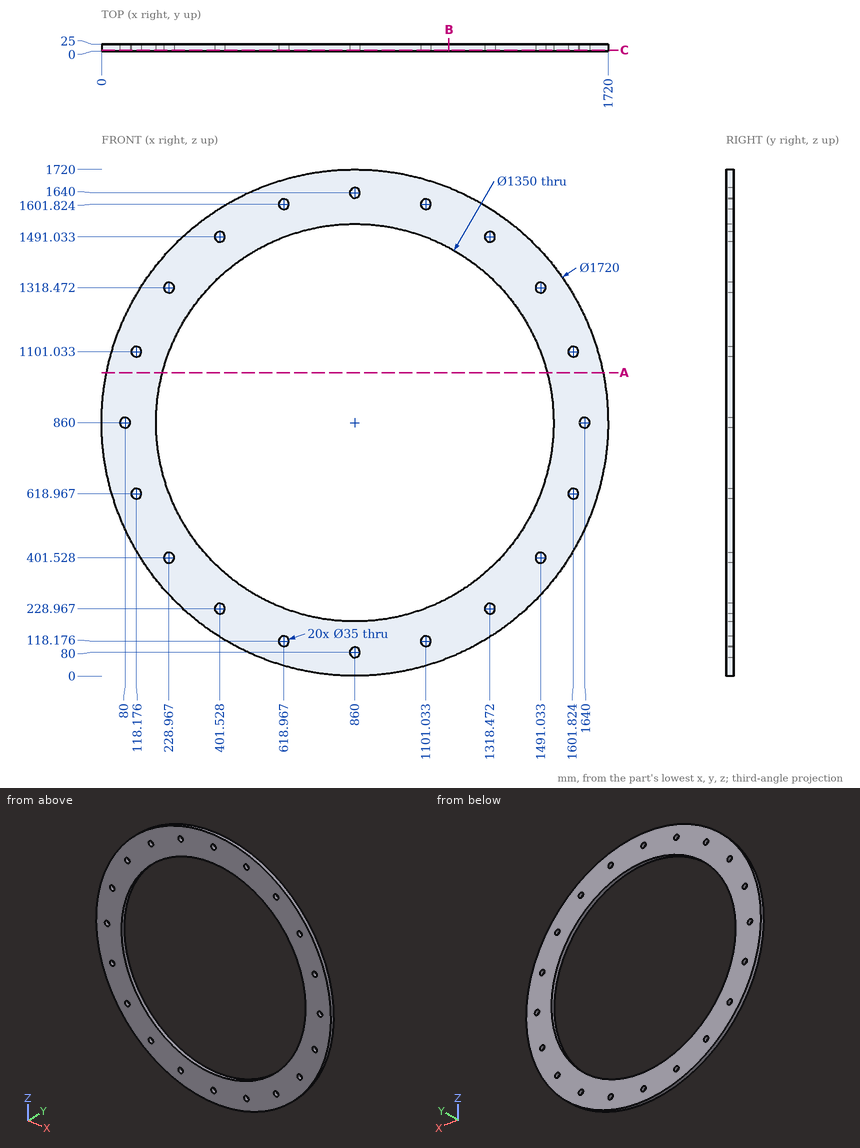
Geometry: see drawing. Coordinates: mm, zero at the bounding-box minimum. Coordinates: 2 decimals unless noted, no trailing zeros. Write each loop counter-clockwise with the first axis right and the second up, starting at its lowest first coordinate (ties: lowest second). Pieces come first, ordered by that corner, then holes. Notation, with made-up numbers: M 36.25,14.5 L 77.25,14.5 A25 ccw 77.25,26.5 Z; hole C 76,36.25 d3. An arc over 180 degrees is marked long. Answer as a JSON object with one key per item and string values.
1. Cut plane C-C on y = 4.25. State how many separate pieces and enclosed holes the cut face has, plus the area to 3 significant figures.
Evaluation:
{"separate pieces": "1", "enclosed holes": "21", "area": "873,000 mm^2"}
2. Ray query, L1, parallel to X at y = 15.25, z = 860; L2, parallel to Z at x = 878, y = 6.75; L3, parallel to Z at x = 1208, y = 9.75 (1 decimal). Return the intervals inside material, ascending.
Evaluation:
{"L1": "0 to 62.5, 97.5 to 185, 1535 to 1622.5, 1657.5 to 1720", "L2": "0.19 to 185.24, 1534.76 to 1719.81", "L3": "73.6 to 281.6, 1438.4 to 1646.4"}
3. Cut plane B-B on x = 1179. Output: boundary loops of the cut face in (y, z) (1 decimal).
Evaluation:
{"outline": "M 0,61.4 L 25,61.4 L 25,265.1 L 0,265.1 Z; M 0,1454.9 L 25,1454.9 L 25,1658.6 L 0,1658.6 Z"}
4. Cut plane A-A on z = 1030. Output: boundary loops of the cut face in (x, y).
Evaluation:
{"outline": "M 16.97,0 L 206.76,0 L 206.76,25 L 16.97,25 Z; M 1513.24,0 L 1703.03,0 L 1703.03,25 L 1513.24,25 Z"}
5. Contact query for flat-ended pins moving along their axis: P1, Ø1.5, axis at x = 222, y = 21, coming from the -Z side (1 decimal); P2, Ø1, axis at x = 599, y = 5.5, coming from the -Z side; P3, Ø3, axis at y = 7, z = 573, coming from the -X side; P4, Ø21, axis at x = 1318.47, z = 1491.03, coming from the +Y side. Output: stop coordinate, or through.
Evaluation:
{"P1": "z = 282.5", "P2": "z = 40.4", "P3": "x = 48.77", "P4": "through"}
